Input: part model. Units: mm. Frame: model coordinates. Face numbers are marked on the shaded views. Give positions to 0.01 mm unless a question says otherwise; leave off trailing zeros. Order: outer loops, then holes, each group sorted by start corner. A loop starts at its lowest first (then second) coordinate and runs counter-clockwise, first axis right, second up. Notation, with made-up numbers: M -14.5,78 L -4.5,78 A37 ccw -4.5,116 Z; hole C 6,30.25 d6. An arc over 180 degrees is marked long. Use a Markdown table: item, result.
from build123d import *

# Parameters (mm, degrees)
SKETCH1_R           = 7
BOSS_EXTRUDE1_DEPTH = 8


with BuildPart() as part:
    # Sketch1 → Boss-Extrude1 (new body)
    with BuildSketch(Plane(origin=(0, 0, 0), x_dir=(1, 0, 0), z_dir=(0, 1, 0))):
        with BuildLine():
            Line((-30, -50), (20, -50))
            ThreePointArc((20, -50), (27.071067812, -47.071067812), (30, -40))
            Line((30, -40), (30, 40))
            ThreePointArc((30, 40), (27.071067812, 47.071067812), (20, 50))
            Line((20, 50), (-30, 50))
            Line((-30, 50), (-30, -50))
        make_face()
        with Locations(Location((10, 30, 0), (0, 0, 270))):
            Circle(SKETCH1_R, mode=Mode.SUBTRACT)
        with Locations(Location((10, -30, 0), (0, 0, 90))):
            Circle(SKETCH1_R, mode=Mode.SUBTRACT)
    extrude(amount=BOSS_EXTRUDE1_DEPTH)


solid = part.part
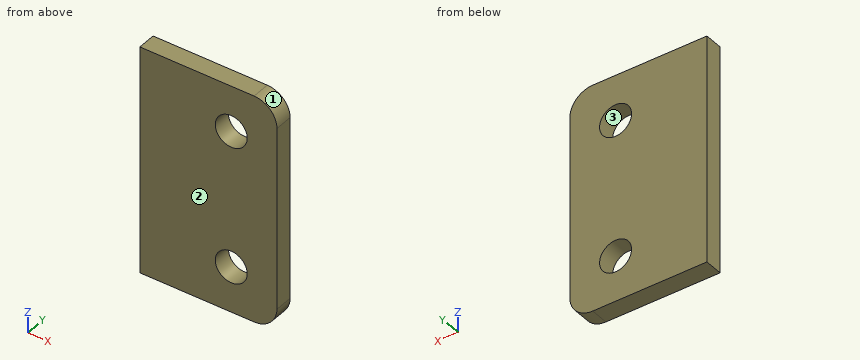
1) Mould query, pull axis Z, two halves, no side actions, for the marked faces 1, 2 and 3. Classes: released by +Z, released by -Z, zero draft, split by the parting line, or undercut.
Response values:
| item | result |
|---|---|
| face 1 | released by +Z |
| face 2 | zero draft |
| face 3 | undercut |
2) Cut plane B-B on y = 6.25. Return loops of the section in (x, z).
Response values:
| item | result |
|---|---|
| outline | M -30,-50 L 20,-50 A10 ccw 30,-40 L 30,40 A10 ccw 20,50 L -30,50 Z; hole C 10,-30 d14; hole C 10,30 d14 |
3) Material intervals for line 1 (X direction, y = 5.75, z = 30); line 2 (Z direction, x = 4, y = 4.25); line 3 (Z direction, x = 8.5, y = 0.75), sorted ascending. Write a range as from..to.
Response values:
| item | result |
|---|---|
| line 1 | x = -30..3, 17..30 |
| line 2 | z = -50..-33.61, -26.39..26.39, 33.61..50 |
| line 3 | z = -50..-36.84, -23.16..23.16, 36.84..50 |
4) First-contact query: pin 1 Ø8.5 at (x, z) = (10, -30) entering from -Y. Flat tip, straight axial feed; report the tip coordinate or a pass-through.
Response values:
| item | result |
|---|---|
| pin 1 | passes through |
5) Cut plane C-C on z = -30. Return loops of the section in (x, y).
Response values:
| item | result |
|---|---|
| outline | M -30,0 L 3,0 L 3,8 L -30,8 Z; M 17,0 L 30,0 L 30,8 L 17,8 Z |
6) Cut plane A-A on x = 10. Return loops of the section in (y, z).
Response values:
| item | result |
|---|---|
| outline | M 0,-50 L 8,-50 L 8,-37 L 0,-37 Z; M 0,-23 L 8,-23 L 8,23 L 0,23 Z; M 0,37 L 8,37 L 8,50 L 0,50 Z |
7) Cut plane D-D on x = 4. Return loops of the section in (y, z).
Response values:
| item | result |
|---|---|
| outline | M 0,-50 L 8,-50 L 8,-33.61 L 0,-33.61 Z; M 0,-26.39 L 8,-26.39 L 8,26.39 L 0,26.39 Z; M 0,33.61 L 8,33.61 L 8,50 L 0,50 Z |
